Geometry: final body of the model. Coordinates: model frame, mm. A direction names the side the tool comes from. Coordinates: 2 decimals unless noted, no trailing zeros. Order: outer loops, then holes, each group sorted by start corner. A loop starts at its lowest first (then second) coordinate and runs counter-clockwise, first axis right, second up. Notation, with made-up numbers: (43, 59) - (90, 59) arc R19 ccw to (90, 69) - close; hole circle Ø11 at (66, -11.5). An arc over 180 degrees is marked (long way). Use a Markdown table: item, result. Add a question column.
```python
from build123d import *

# Parameters (mm, degrees)
SKETCH1_R                 = 2.65
F_30_X_60G_X_R1_5_1_DEPTH = 450


with BuildPart() as part:
    # Sketch1 → 工业铝型材 30 X 60G X R1.5(1) (new body)
    with BuildSketch(Plane(origin=(0, 0, 0), x_dir=(-1, 0, 0), z_dir=(0, 1, 0))):
        with BuildLine():
            Line((-3.25, 30), (-3.25, 29))
            Line((-3.25, 29), (-4.25, 29))
            Line((-4.25, 29), (-4.25, 21.277812156))
            ThreePointArc((-4.25, 21.277812156), (0, 20.5), (4.25, 21.277812156))
            Line((4.25, 21.277812156), (4.25, 29))
            Line((4.25, 29), (3.25, 29))
            Line((3.25, 29), (3.25, 30))
            Line((3.25, 30), (13.5, 30))
            ThreePointArc((13.5, 30), (14.560660172, 29.560660172), (15, 28.5))
            Line((15, 28.5), (15, 18.25))
            Line((15, 18.25), (14, 18.25))
            Line((14, 18.25), (14, 19.25))
            Line((14, 19.25), (6.277812156, 19.25))
            ThreePointArc((6.277812156, 19.25), (5.5, 15), (6.277812156, 10.75))
            Line((6.277812156, 10.75), (14, 10.75))
            Line((14, 10.75), (14, 11.75))
            Line((14, 11.75), (15, 11.75))
            Line((15, 11.75), (15, -11.75))
            Line((15, -11.75), (14, -11.75))
            Line((14, -11.75), (14, -10.75))
            Line((14, -10.75), (6.277812156, -10.75))
            ThreePointArc((6.277812156, -10.75), (5.5, -15), (6.277812156, -19.25))
            Line((6.277812156, -19.25), (14, -19.25))
            Line((14, -19.25), (14, -18.25))
            Line((14, -18.25), (15, -18.25))
            Line((15, -18.25), (15, -28.5))
            ThreePointArc((15, -28.5), (14.560660172, -29.560660172), (13.5, -30))
            Line((13.5, -30), (3.25, -30))
            Line((3.25, -30), (3.25, -29))
            Line((3.25, -29), (4.25, -29))
            Line((4.25, -29), (4.25, -21.277812156))
            ThreePointArc((4.25, -21.277812156), (0, -20.5), (-4.25, -21.277812156))
            Line((-4.25, -21.277812156), (-4.25, -29))
            Line((-4.25, -29), (-3.25, -29))
            Line((-3.25, -29), (-3.25, -30))
            Line((-3.25, -30), (-13.5, -30))
            ThreePointArc((-13.5, -30), (-14.560660172, -29.560660172), (-15, -28.5))
            Line((-15, -28.5), (-15, -18.25))
            Line((-15, -18.25), (-14, -18.25))
            Line((-14, -18.25), (-14, -19.25))
            Line((-14, -19.25), (-6.277812156, -19.25))
            ThreePointArc((-6.277812156, -19.25), (-5.5, -15), (-6.277812156, -10.75))
            Line((-6.277812156, -10.75), (-14, -10.75))
            Line((-14, -10.75), (-14, -11.75))
            Line((-14, -11.75), (-15, -11.75))
            Line((-15, -11.75), (-15, 11.75))
            Line((-15, 11.75), (-14, 11.75))
            Line((-14, 11.75), (-14, 10.75))
            Line((-14, 10.75), (-6.277812156, 10.75))
            ThreePointArc((-6.277812156, 10.75), (-5.5, 15), (-6.277812156, 19.25))
            Line((-6.277812156, 19.25), (-14, 19.25))
            Line((-14, 19.25), (-14, 18.25))
            Line((-14, 18.25), (-15, 18.25))
            Line((-15, 18.25), (-15, 28.5))
            ThreePointArc((-15, 28.5), (-14.560660172, 29.560660172), (-13.5, 30))
            Line((-13.5, 30), (-3.25, 30))
        make_face()
        with Locations((-11, 26)):
            Circle(SKETCH1_R, mode=Mode.SUBTRACT)
        with Locations((11, 26)):
            Circle(SKETCH1_R, mode=Mode.SUBTRACT)
        with Locations((11, -26)):
            Circle(SKETCH1_R, mode=Mode.SUBTRACT)
        with Locations((-11, -26)):
            Circle(SKETCH1_R, mode=Mode.SUBTRACT)
        with BuildLine():
            Line((-12.5, 7.5), (-4, 7.5))
            Line((-4, 7.5), (-1.665625283, 13.135679101))
            ThreePointArc((-1.665625283, 13.135679101), (0, 17.5), (1.665625283, 13.135679101))
            Line((1.665625283, 13.135679101), (4, 7.5))
            Line((4, 7.5), (12.5, 7.5))
            Line((12.5, 7.5), (12.5, -7.5))
            Line((12.5, -7.5), (4, -7.5))
            Line((4, -7.5), (1.665625283, -13.135679101))
            ThreePointArc((1.665625283, -13.135679101), (0, -17.5), (-1.665625283, -13.135679101))
            Line((-1.665625283, -13.135679101), (-4, -7.5))
            Line((-4, -7.5), (-12.5, -7.5))
            Line((-12.5, -7.5), (-12.5, 7.5))
        make_face(mode=Mode.SUBTRACT)
    extrude(amount=F_30_X_60G_X_R1_5_1_DEPTH)


solid = part.part
```
1) Section query B-B (y = 364). Give the number of separate pieces and of enclosed holes in the cut face, and give its area (3 significant figures).
2) First-contact query: pin 1 (1.1 mm diameter, centred on x = -14.5, y = 305, fed in from -Z); pin 2 (1 mm diameter, centred on x = 0, y = 400.5, fed in from -Z). Flat tips, straight axial feed; report the tip coordinate or a pass-through.
3) Access query for faces 5 (the flat face through (-12.5, 222, 0)), 6 (the flat face through (15, 222, 0)). Directions: +Z, -Z, +X, -X, +Y, -Y. A direction counts if a zero-diameter tool reaches every point of the face in a straight line with its end or side. Return the directions, or none.
4) Draft query along X for faces 1 (the flat face through (8, 222, 7.5)), 2 (the flat face through (8, 222, 30)), 3 (the flat face through (-15, 222, 23)), 4 (the flat face through (10, 222, 19.25)). Return one class per face: released by +X, released by -X, zero draft, split by the parting line, or undercut.
5) Line query: line 1 (Z direction, x = -4, y = 400); line 2 (Z direction, x = 7.75, y = 101.5); line 3 (Z direction, x = -11, y = 176.5). Output: solid intervals per line, ascending. Write a range as from..to.
6) Section query A-A (z = -3). Return the cut outline in (x, y).
From the geometry:
| question | item | result |
|---|---|---|
| 1 | separate pieces | 1 |
| 1 | enclosed holes | 5 |
| 1 | area | 775 mm^2 |
| 2 | pin 1 | stops at z = -29.93 |
| 2 | pin 2 | stops at z = -20.51 |
| 3 | face 5 | +Y, -Y |
| 3 | face 6 | +Z, -Z, +X, +Y, -Y |
| 4 | face 1 | undercut |
| 4 | face 2 | zero draft |
| 4 | face 3 | released by -X |
| 4 | face 4 | undercut |
| 5 | line 1 | z = -30..-29, -21.19..-7.5, 7.5..21.19, 29..30 |
| 5 | line 2 | z = -30..-19.25, -10.75..-7.5, 7.5..10.75, 19.25..30 |
| 5 | line 3 | z = -30..-28.65, -23.35..-19.25, -10.75..-7.5, 7.5..10.75, 19.25..23.35, 28.65..30 |
| 6 | outline | (-15, 0) - (-12.5, 0) - (-12.5, 450) - (-15, 450) - close; (12.5, 0) - (15, 0) - (15, 450) - (12.5, 450) - close |
